from build123d import *

# Parameters (mm, degrees)
SKETCH1_R           = 1.75
SKETCH1_R_2         = 2
BOSS_EXTRUDE1_DEPTH = 2
CHAMFER1_SIZE       = 1
SKETCH3_R           = 2.9
BOSS_EXTRUDE2_DEPTH = 15
CHAMFER2_SIZE       = 0.5


with BuildPart() as part:
    # Sketch1 → Boss-Extrude1 (new body)
    with BuildSketch(Plane(origin=(0, 0, 0), x_dir=(1, 0, 0), z_dir=(0, 1, 0))):
        with BuildLine():
            Line((-104.75, -124.75), (104.75, -124.75))
            ThreePointArc((104.75, -124.75), (118.892135624, -118.892135624), (124.75, -104.75))
            Line((124.75, -104.75), (124.75, 104.75))
            ThreePointArc((124.75, 104.75), (118.892135624, 118.892135624), (104.75, 124.75))
            Line((104.75, 124.75), (-104.75, 124.75))
            ThreePointArc((-104.75, 124.75), (-118.892135624, 118.892135624), (-124.75, 104.75))
            Line((-124.75, 104.75), (-124.75, -104.75))
            ThreePointArc((-124.75, -104.75), (-118.892135624, -118.892135624), (-104.75, -124.75))
        make_face()
        with Locations(Location((-90, 106.75, 0), (0, 0, 270))):
            Circle(SKETCH1_R, mode=Mode.SUBTRACT)
        with Locations(Location((0, 106.75, 0), (0, 0, 270))):
            Circle(SKETCH1_R, mode=Mode.SUBTRACT)
        with Locations(Location((90, 106.75, 0), (0, 0, 270))):
            Circle(SKETCH1_R, mode=Mode.SUBTRACT)
        with Locations(Location((106.75, 90, 0), (0, 0, 270))):
            Circle(SKETCH1_R, mode=Mode.SUBTRACT)
        with Locations(Location((106.75, 0, 0), (0, 0, 270))):
            Circle(SKETCH1_R, mode=Mode.SUBTRACT)
        with Locations(Location((106.75, -90, 0), (0, 0, 270))):
            Circle(SKETCH1_R, mode=Mode.SUBTRACT)
        with Locations(Location((90, -106.75, 0), (0, 0, 270))):
            Circle(SKETCH1_R, mode=Mode.SUBTRACT)
        with Locations(Location((0, -106.75, 0), (0, 0, 270))):
            Circle(SKETCH1_R, mode=Mode.SUBTRACT)
        with Locations(Location((-90, -106.75, 0), (0, 0, 270))):
            Circle(SKETCH1_R, mode=Mode.SUBTRACT)
        with Locations(Location((-106.75, -90, 0), (0, 0, 270))):
            Circle(SKETCH1_R, mode=Mode.SUBTRACT)
        with Locations(Location((-106.75, 0, 0), (0, 0, 270))):
            Circle(SKETCH1_R, mode=Mode.SUBTRACT)
        with Locations(Location((-106.75, 90, 0), (0, 0, 270))):
            Circle(SKETCH1_R, mode=Mode.SUBTRACT)
        with Locations(Location((0, 0, 0), (0, 0, 270))):
            Circle(SKETCH1_R_2, mode=Mode.SUBTRACT)
    extrude(amount=BOSS_EXTRUDE1_DEPTH)

    # Chamfer1
    chamfer1_edges = [part.edges().sort_by_distance(p)[0] for p in [
        (-90, 2, -108.5),
        (0, 2, -108.5),
        (90, 2, -108.5),
        (106.75, 2, -91.75),
        (106.75, 2, -1.75),
        (106.75, 2, 88.25),
        (90, 2, 105),
        (0, 2, 105),
        (-90, 2, 105),
        (-106.75, 2, 88.25),
        (-106.75, 2, -1.75),
        (-106.75, 2, -91.75),
    ]]
    chamfer(chamfer1_edges, length=CHAMFER1_SIZE)

    # Sketch3 → Boss-Extrude2 (add)
    with BuildSketch(Plane(origin=(0, 2, 0), x_dir=(1, 0, 0), z_dir=(0, 1, 0))):
        with Locations(Location((-18.03122292, -20, 0), (0, 0, 90))):
            Circle(SKETCH3_R)
        with Locations(Location((18.03122292, -20, 0), (0, 0, 90))):
            Circle(SKETCH3_R)
        with Locations(Location((18.03122292, -56.062445841, 0), (0, 0, 90))):
            Circle(SKETCH3_R)
        with Locations(Location((-18.03122292, -56.062445841, 0), (0, 0, 90))):
            Circle(SKETCH3_R)
    extrude(amount=BOSS_EXTRUDE2_DEPTH)

    # Chamfer2
    chamfer2_edges = [part.edges().sort_by_distance(p)[0] for p in [
        (-18.03122292, 17, 22.9),
        (18.03122292, 17, 22.9),
        (18.03122292, 17, 58.962445841),
        (-18.03122292, 17, 58.962445841),
    ]]
    chamfer(chamfer2_edges, length=CHAMFER2_SIZE)


solid = part.part
Read the model definition and answer for the solid it produces. Units are mm, in the model's axes. A direction names the side the tool comes from. Round coordinates to 2 decimals unless told otherwise and drop trailing zeros. Order: outer loops, then holes, each group sorted by start corner. A loop starts at its lowest first (then second) coordinate and runs counter-clockwise, first axis right, second up.
1) For faces 1 (the face through (-16.921, 9.148, 53.384)), 2 (the face through (-119.047, 0.986, 118.736)), determine the directions among +Z, -Z, +X, -X, +Y, -Y from which every point of the face is accessible in a straight line to the end or side of a thin tool.
2) Flat-ended cylindrical pins translate along their axes: pin 1 (4.5 mm diameter, centred on x = -106.75, z = -90, fed in from +Y); pin 2 (2 mm diameter, centred on x = 106.75, z = -90, fed in from +Y) (3 decimals); pin 3 (3 mm diameter, centred on x = -89.5, z = -51, fed in from +Y); pin 4 (4 mm diameter, centred on x = -90, z = -106.75, fed in from +Y). Find the tip coordinate at first contact, or state that the pin passes through.
3) The part is cut by section A-A on y = 5. Write down the section's boundary in (x, z), plus the area to 3 significant figures.
4) The part is cut by section B-B on x = 73.5. Write down the section's boundary in (y, z).
5) The part is cut by section C-C on z = 83.5. Write down the section's boundary in (x, y), plus the area to 3 significant figures.
6) The mould has two halves that part along X. Classify faces 3 (the face through (-118.736, 0.986, -119.047)), 4 (the face through (119.047, 0.986, -118.736)), 5 (the face through (19.8, 9.1, 22.3)): released by +X, released by -X, zero draft, split by the parting line, or undercut.
7) Straight lines are drawn through the part: L1, parallel to X at y = 0.3, z = 0; L2, parallel to Z at x = -90, y = 0.75; L3, parallel to Z at x = -106.75, y = 0.45. For each, find the intervals that lie inside material, in ascending order.
Resolved:
1. face 1: +Y
1. face 2: +Z, -X, +Y, -Y
2. pin 1: stops at y = 1.5
2. pin 2: passes through
2. pin 3: stops at y = 2
2. pin 4: stops at y = 1.25
3. outline: circle Ø5.8 at (-18.03, 20); circle Ø5.8 at (-18.03, 56.06); circle Ø5.8 at (18.03, 20); circle Ø5.8 at (18.03, 56.06)
3. area: 106 mm2
4. outline: (0, -124.75) - (2, -124.75) - (2, 124.75) - (0, 124.75) - close
5. outline: (-124.75, 0) - (124.75, 0) - (124.75, 2) - (-124.75, 2) - close
5. area: 499 mm2
6. face 3: released by -X
6. face 4: released by +X
6. face 5: undercut
7. L1: x = -124.75 to -108.5, -105 to -2, 2 to 105, 108.5 to 124.75
7. L2: z = -124.75 to -108.5, -105 to 105, 108.5 to 124.75
7. L3: z = -124.65 to -91.75, -88.25 to -1.75, 1.75 to 88.25, 91.75 to 124.65
